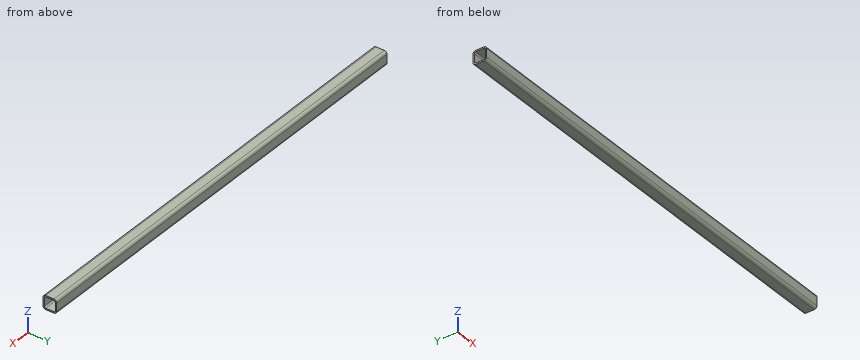
```python
from build123d import *

# Parameters (mm, degrees)
SQUARE_TUBE_40_X_40_X_4_1_DEPTH = 1280


with BuildPart() as part:
    # Sketch1 → Square Tube 40 X 40 X 4(1) (new body)
    with BuildSketch(Plane.YZ.offset(-1000)):
        with BuildLine():
            Line((-12, -20), (12, -20))
            ThreePointArc((12, -20), (17.656854249, -17.656854249), (20, -12))
            Line((20, -12), (20, 12))
            ThreePointArc((20, 12), (17.656854249, 17.656854249), (12, 20))
            Line((12, 20), (-12, 20))
            ThreePointArc((-12, 20), (-17.656854249, 17.656854249), (-20, 12))
            Line((-20, 12), (-20, -12))
            ThreePointArc((-20, -12), (-17.656854249, -17.656854249), (-12, -20))
        make_face()
        with BuildLine():
            Line((-12, -16), (12, -16))
            ThreePointArc((12, -16), (14.828427125, -14.828427125), (16, -12))
            Line((16, -12), (16, 12))
            ThreePointArc((16, 12), (14.828427125, 14.828427125), (12, 16))
            Line((12, 16), (-12, 16))
            ThreePointArc((-12, 16), (-14.828427125, 14.828427125), (-16, 12))
            Line((-16, 12), (-16, -12))
            ThreePointArc((-16, -12), (-14.828427125, -14.828427125), (-12, -16))
        make_face(mode=Mode.SUBTRACT)
    extrude(amount=SQUARE_TUBE_40_X_40_X_4_1_DEPTH)


solid = part.part
```
The model under review builds one solid part; all positions refer to its coordinate system, in mm. Give positions to 0.01 mm unless a question says otherwise; leave off trailing zeros. Write each loop counter-clockwise with the first axis right and the second up, starting at its lowest first coordinate (ties: lowest second). Pieces come first, ordered by that corner, then holes. Notation, with made-up numbers: M 24.25,-0.75 L 29.25,-0.75 A28 cw 29.25,19.25 Z; hole C -39,25 d8. An arc over 180 degrees is marked long. Write each question's results on one line, items separated by ' | '. Start each with the question number.
1. For probe 1 along Z at (x, y) = (-72, -2.5); probe 2 along Z at (x, y) = (-880, -14.5), list the stretches that pass through material, from the lowest coordinate up. Write a range as [from, to].
2. We need section A-A (z = -2.5). Write out the cut boundary in (x, y), and give its area (3 significant figures).
3. Insertion check: pin 1 Ø4 at (y, z) = (7, -12.5) entering from +X; pin 2 Ø1 at (x, z) = (-48, 16) entering from -Y. Each pin has a flat end and moves straight along its axis. Give the tip position at first contact, or say it passes through.
4. We need section C-C (x = -197). Write out the cut boundary in (y, z), and give its area (3 significant figures).
Results found:
1) probe 1: z = [-20, -16], [16, 20] | probe 2: z = [-19.6, -15.12], [15.12, 19.6]
2) outline: M -1000,-20 L 280,-20 L 280,-16 L -1000,-16 Z; M -1000,16 L 280,16 L 280,20 L -1000,20 Z | area: 10,200 mm^2
3) pin 1: passes through | pin 2: stops at y = -19.19
4) outline: M -20,-12 A8 ccw -12,-20 L 12,-20 A8 ccw 20,-12 L 20,12 A8 ccw 12,20 L -12,20 A8 ccw -20,12 Z; hole M -16,-12 A4 ccw -12,-16 L 12,-16 A4 ccw 16,-12 L 16,12 A4 ccw 12,16 L -12,16 A4 ccw -16,12 Z | area: 535 mm^2
